Study the drawing (mm; zero at the part's minimum x, y, z) and answer. Round coordinates to 2 decimals unless told otherwise and drop trailing zeros. Loops run counter-clockwise (first coordinate to the right, second up) from the corner with the lowest first, then second, coordinate; pieces in that order, holes last. Notation, with made-up numbers: (68.25, 21) - (80.25, 21) arc R22 cw to (80.25, 56) - close; hole circle Ø9 at (76.25, 32.25). An arc over 180 degrees is marked (long way). One line per item, written item: value.
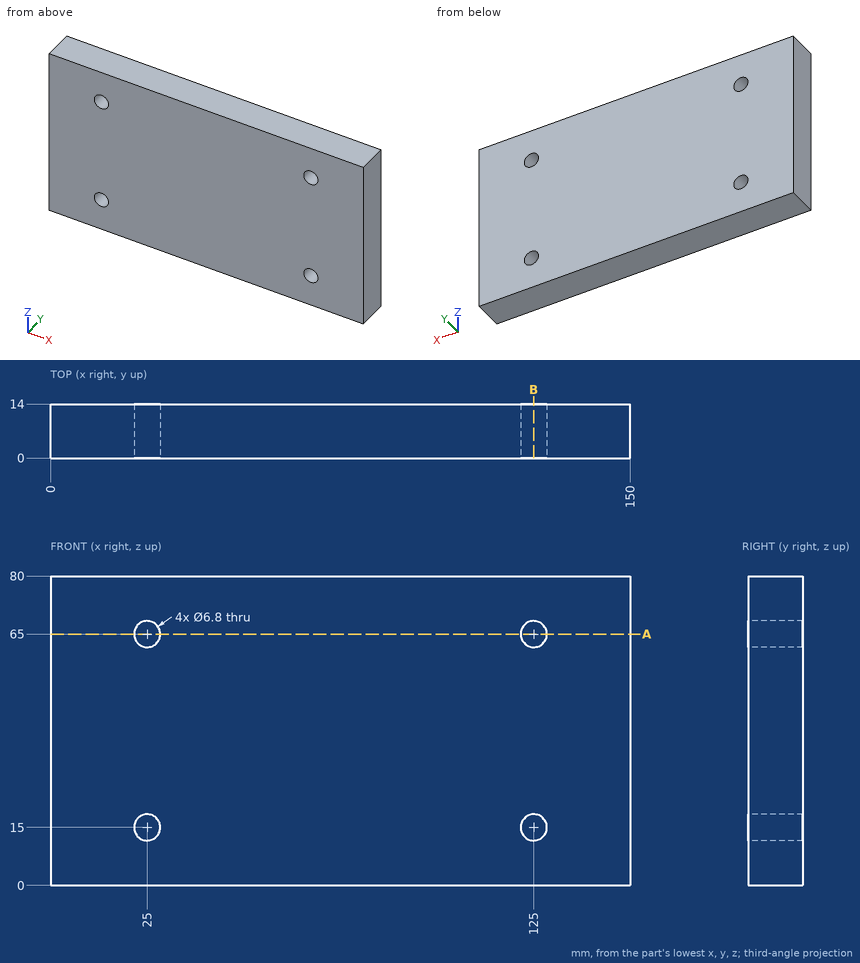
1) A cutting plane is placed at A-A on z = 65. Give the vertices of the cut face in (x, y), and give its area (3 significant figures).
Final values:
outline: (0, 0) - (21.6, 0) - (21.6, 14) - (0, 14) - close; (28.4, 0) - (121.6, 0) - (121.6, 14) - (28.4, 14) - close; (128.4, 0) - (150, 0) - (150, 14) - (128.4, 14) - close
area: 1,910 mm2
2) This flat-tipped pin is pushed along its axis until it touches: pin 1 Ø5.5 at (x, z) = (125, 15) entering from -Y. Where does it stop, or does it pass through?
Final values:
pin 1: through
3) Consider L1, parallel to Z at x = 125, y = 6; L2, parallel to X at y = 11, z = 64. Determine where each line is inside the solid, lowest interval first.
Final values:
L1: 0 to 11.6, 18.4 to 61.6, 68.4 to 80
L2: 0 to 21.75, 28.25 to 121.75, 128.25 to 150
4) A cutting plane is placed at B-B on x = 125. Give the vertices of the cut face in (y, z).
Final values:
outline: (0, 0) - (14, 0) - (14, 11.6) - (0, 11.6) - close; (0, 18.4) - (14, 18.4) - (14, 61.6) - (0, 61.6) - close; (0, 68.4) - (14, 68.4) - (14, 80) - (0, 80) - close
